Read the model definition and answer for the solid it produces. Units are mm, in the model's axes. A direction names the side the tool comes from. Coordinates: 2 decimals unless noted, no trailing zeros. Write each loop counter-clockwise with the first axis right and the second up, starting at its lowest first coordinate (ties: lowest second). Pieces come first, ordered by that corner, then holes.
from build123d import *

# Parameters (mm, degrees)
GB_T_707_1988_HOT_ROLLED_CHANNEL_05_1_DEPTH = 454


with BuildPart() as part:
    # Sketch1 → GB/T 707-1988 hot-rolled channel 05(1) (new body)
    with BuildSketch(Plane.YZ.offset(-227)):
        with BuildLine():
            Line((37, 50), (0, 50))
            Line((0, 50), (0, 0))
            Line((0, 0), (37, 0))
            Line((37, 0), (37, 2.140642022))
            ThreePointArc((37, 2.140642022), (36.101006889, 4.482599144), (33.865849621, 5.621468656))
            Line((33.865849621, 5.621468656), (10.768300757, 8.049118866))
            ThreePointArc((10.768300757, 8.049118866), (6.297986222, 10.326857889), (4.5, 15.010772133))
            Line((4.5, 15.010772133), (4.5, 34.989227867))
            ThreePointArc((4.5, 34.989227867), (6.297986222, 39.673142111), (10.768300757, 41.950881134))
            Line((10.768300757, 41.950881134), (33.865849621, 44.378531344))
            ThreePointArc((33.865849621, 44.378531344), (36.101006889, 45.517400856), (37, 47.859357978))
            Line((37, 47.859357978), (37, 50))
        make_face()
    extrude(amount=GB_T_707_1988_HOT_ROLLED_CHANNEL_05_1_DEPTH)


solid = part.part
Item 1: Given pin 1 (10 mm diameter, centred on y = 6.5, z = 38.5, fed in from +X); pin 2 (22 mm diameter, centred on x = 64.5, z = 22, fed in from +Y), each flat-ended and moving along its own axis, determine where each tip first touches the part or whether it passes through.
Item 2: The part is cut by section C-C (z = 21). Give the vertices of the cut face in (x, y).
Item 3: Find the intervals of material crossed by probe 1 along Y at (x, z) = (71.5, 17); probe 2 along Z at (x, y) = (-135, 24); probe 3 along Z at (x, y) = (179, 30.5), in increasing order.
Item 4: For faces 5 (the cylindrical face through (-3.18, 6.35, 10.27)), 6 (the flat face through (-3, 19, 50)), determine the directions among +Z, -Z, +X, -X, +Y, -Y from which every point of the face is accessible in a straight line to the end or side of a thin tool.
Item 5: Determine the mould class of faces 1 (the flat face through (227, 3, 23)), 2 (the flat face through (-3, 4.5, 25)), 3 (the flat face through (-3, 18, 0)), 4 (the cylindrical face through (-3.18, 6.25, 39.62)) for opening direction Z: +Z half, -Z half, draft (parallel to the pull), parting line (faces both ways), or undercut.
Item 6: The part is cut by section B-B (x = -140). Give the vertices of the cut face in (y, z), and give its area (3 significant figures).
Item 7: The part is cut by section A-A (y = 29). Give the vertices of the cut face in (x, z).
Answer:
1. pin 1: stops at x = 227
1. pin 2: stops at y = 5.76
2. outline: (-227, 0) - (227, 0) - (227, 4.5) - (-227, 4.5) - close
3. probe 1: y = 0 to 4.5
3. probe 2: z = 0 to 6.66, 43.34 to 50
3. probe 3: z = 0 to 5.98, 44.02 to 50
4. face 5: +X, -X, +Y
4. face 6: +Z, +X, -X, +Y, -Y
5. face 1: draft
5. face 2: undercut
5. face 3: -Z half
5. face 4: undercut
6. outline: (0, 0) - (37, 0) - (37, 2.14) arc R3.5 ccw to (33.87, 5.62) - (10.77, 8.05) arc R7 cw to (4.5, 15.01) - (4.5, 34.99) arc R7 cw to (10.77, 41.95) - (33.87, 44.38) arc R3.5 ccw to (37, 47.86) - (37, 50) - (0, 50) - close
6. area: 692 mm2
7. outline: (-227, 0) - (227, 0) - (227, 6.13) - (-227, 6.13) - close; (-227, 43.87) - (227, 43.87) - (227, 50) - (-227, 50) - close
